```python
from build123d import *

# Parameters (mm, degrees)
SKETCH1_W                                            = 480
SKETCH1_H                                            = 20
BOSS_EXTRUDE1_DEPTH                                  = 10
HOLE_SIZE_PER_SOCKET_HEAD_CAP_SCREW_TYPE_D           = 5.5
HOLE_SIZE_PER_SOCKET_HEAD_CAP_SCREW_TYPE_CBORE_D     = 10
HOLE_SIZE_PER_SOCKET_HEAD_CAP_SCREW_TYPE_CBORE_DEPTH = 5.7
CHAMFER1_SIZE                                        = 1
F_4_0_4_DIAMETER_HOLE1_D                             = 4
F_4_0_4_DIAMETER_HOLE1_DEPTH                         = 12
F_4_0_4_DIAMETER_HOLE1_TIP                           = 1.201721238


with BuildPart() as part:
    # Sketch1 → Boss-Extrude1 (new body)
    with BuildSketch(Plane.XY):
        Rectangle(SKETCH1_W, SKETCH1_H)
    extrude(amount=BOSS_EXTRUDE1_DEPTH)

    # Hole size per socket head cap screw type1 (through all)
    with Locations(Plane.XY.offset(10)):
        with Locations((0, 0), (-110, 0), (110, 0), (220, 0), (-220, 0)):
            CounterBoreHole(HOLE_SIZE_PER_SOCKET_HEAD_CAP_SCREW_TYPE_D / 2, HOLE_SIZE_PER_SOCKET_HEAD_CAP_SCREW_TYPE_CBORE_D / 2, HOLE_SIZE_PER_SOCKET_HEAD_CAP_SCREW_TYPE_CBORE_DEPTH)

    # Chamfer1
    chamfer1_edges = [part.edges().sort_by_distance(p)[0] for p in [
        (240, -10, 5),
        (-240, -10, 5),
        (-240, 10, 5),
        (240, 10, 5),
    ]]
    chamfer(chamfer1_edges, length=CHAMFER1_SIZE)

    # Ø4.0 (4) Diameter Hole1
    with Locations(Plane.XY.offset(10)):
        with Locations((-150, 0), (150, 0)):
            Hole(F_4_0_4_DIAMETER_HOLE1_D / 2, depth=F_4_0_4_DIAMETER_HOLE1_DEPTH)
            with Locations((0, 0, -(F_4_0_4_DIAMETER_HOLE1_DEPTH + F_4_0_4_DIAMETER_HOLE1_TIP / 2))):  # 118° drill point
                Cone(0, F_4_0_4_DIAMETER_HOLE1_D / 2, F_4_0_4_DIAMETER_HOLE1_TIP, mode=Mode.SUBTRACT)


solid = part.part
```
Here's how the part is built. I have some questions about the finished solid (model axes, mm). A direction names the side the tool comes from. Give positions to 0.01 mm unless a question says otherwise; leave off trailing zeros. Loops run counter-clockwise (first coordinate to the right, second up) from the corner with the lowest first, then second, coordinate; pieces in that order, holes last. Notation, with made-up numbers: M 48.25,31 L 95.25,31 A14 cw 95.25,48 Z; hole C -36.5,81.5 d11. An arc over 180 degrees is marked long. Put each result on its own line as item: value. Start each with the question number.
(1) I need wall thicknesses on line 1 along Y through (x, z) = (0, 1.75); line 2 along Y through (x, z) = (0, 7.95); line 3 along X through (y, z) = (-4.5, 4.75). Which ranges of each line are inside material? Lowest first, please. Write a range as [from, to].
(2) I want a section at A-A on z = 1.5. Please give me the cut outline in (x, y), then the cut area to 3 significant figures.
(3) For faces 5 (the flat face through (2.2, -2.2, 4.3)), 6 (the flat face through (-240, 0, 5)), which set-ups out of +Z, -Z, +X, -X, +Y, -Y let a thin tool reach every point of the face, with its end or its side?
(4) Will these pins go through, and if not, where does the flat tip stop? pin 1 Ø9 at (x, y) = (-220, 0) entering from +Z; pin 2 Ø4.5 at (x, y) = (-220, 0) entering from +Z.
(5) If we mould it in two halves opening along Y, with no side actions, what happens to faces 1 (the flat face through (-3.4, -4.3, 10)), 2 (the flat face through (-3, 10, 5)), 3 (the flat face through (-3, -10, 5)), 4 (the cylindrical face through (-105.381, -1.915, 7.19))? For each: +Y half, -Y half, draft (parallel to the pull), parting line (faces both ways), or undercut.
Answer block:
1. line 1: [-10, -2.75], [2.75, 10]
1. line 2: [-10, -5], [5, 10]
1. line 3: [-240, -222.18], [-217.82, -112.18], [-107.82, -2.18], [2.18, 107.82], [112.18, 217.82], [222.18, 240]
2. outline: M -240,-9 L -239,-10 L 239,-10 L 240,-9 L 240,9 L 239,10 L -239,10 L -240,9 Z; hole C -220,0 d5.5; hole C -150,0 d4; hole C -110,0 d5.5; hole C 0,0 d5.5; hole C 110,0 d5.5; hole C 150,0 d4; hole C 220,0 d5.5
2. area: 9,450 mm^2
3. face 5: +Z
3. face 6: +Z, -Z, -X, +Y, -Y
4. pin 1: z = 4.3
4. pin 2: through
5. face 1: draft
5. face 2: +Y half
5. face 3: -Y half
5. face 4: undercut
